from build123d import *

# Parameters (mm, degrees)
SKETCH1_W           = 20
SKETCH1_H           = 10
SKETCH1_R           = 1.5
BOSS_EXTRUDE1_DEPTH = 0.5


with BuildPart() as part:
    # Sketch1 → Boss-Extrude1 (new body)
    with BuildSketch(Plane(origin=(0, 0, 0), x_dir=(1, 0, 0), z_dir=(0, 1, 0))):
        Rectangle(SKETCH1_W, SKETCH1_H)
        with Locations(Location((-3.5, 0, 0), (0, 0, 270))):
            Circle(SKETCH1_R, mode=Mode.SUBTRACT)
        with Locations(Location((3.5, 0, 0), (0, 0, 90))):
            Circle(SKETCH1_R, mode=Mode.SUBTRACT)
    extrude(amount=BOSS_EXTRUDE1_DEPTH)


solid = part.part
Build history of the part. All positions in model axes, mm. Coordinates: 2 decimals unless noted, no trailing zeros. Order: outer loops, then holes, each group sorted by start corner. A loop starts at its lowest first (then second) coordinate and runs counter-clockwise, first axis right, second up. Notation, with made-up numbers: (25, -1) - (71, -1) arc R22 ccw to (71, 37) - close; hole circle Ø11 at (46, 12.25). An arc over 180 degrees is marked (long way). Put each result on its own line as item: value.
1. Drop a flat-ended pin along its axis: P1, Ø2.5, axis at x = 3.5, z = 0, coming from the -Y side. Give the stop position or say it passes through.
Answer sheet:
P1: passes through
2. Pull direction Z, two halves, no side cores. Call faces 1 (the face through (0, 0, 0)), 2 (the face through (2.013, 0.246, 0.195)): pulls with the +Z half, pulls with the -Z half, needs draft (parallel to the pull), parting line crosses it, or undercut.
Answer sheet:
face 1: needs draft
face 2: undercut
3. Probe line 1 along X through (y, z) = (0.25, 0); line 2 along X through (y, z) = (0.45, 1.25); line 3 along Z through (x, y) = (4.5, 0.05). List the from-to ranges inside material, lowest first. Write a range as [from, to].
Answer sheet:
line 1: x = [-10, -5], [-2, 2], [5, 10]
line 2: x = [-10, -4.33], [-2.67, 2.67], [4.33, 10]
line 3: z = [-5, -1.12], [1.12, 5]
4. Saw through at B-B (x = 3.5). Write the cut outline in (y, z).
Answer sheet:
outline: (0, -5) - (0.5, -5) - (0.5, -1.5) - (0, -1.5) - close; (0, 1.5) - (0.5, 1.5) - (0.5, 5) - (0, 5) - close
5. Saw through at A-A (z = 0). Write the cut outline in (x, y), and give its area (3 significant figures).
Answer sheet:
outline: (-10, 0) - (-5, 0) - (-5, 0.5) - (-10, 0.5) - close; (-2, 0) - (2, 0) - (2, 0.5) - (-2, 0.5) - close; (5, 0) - (10, 0) - (10, 0.5) - (5, 0.5) - close
area: 7.00 mm^2
6. Saw through at C-C (y = 0.2). Write the cut outline in (x, z), and give its area (3 significant figures).
Answer sheet:
outline: (-10, -5) - (10, -5) - (10, 5) - (-10, 5) - close; hole circle Ø3 at (-3.5, 0); hole circle Ø3 at (3.5, 0)
area: 186 mm^2
